from build123d import *

# Parameters (mm, degrees)
SKETCH1_W                                            = 120
SKETCH1_H                                            = 45
BOSS_EXTRUDE1_DEPTH                                  = 12
CHAMFER1_SIZE                                        = 1
SKETCH2_R                                            = 18
CUT_EXTRUDE1_DEPTH                                   = 66.193941436
M4_TAPPED_HOLE1_D                                    = 3.3
HOLE_SIZE_PER_SOCKET_HEAD_CAP_SCREW_TYPE_D           = 6.6
HOLE_SIZE_PER_SOCKET_HEAD_CAP_SCREW_TYPE_CBORE_D     = 11
HOLE_SIZE_PER_SOCKET_HEAD_CAP_SCREW_TYPE_CBORE_DEPTH = 6.8
SKETCH7_R                                            = 6
CUT_EXTRUDE2_DEPTH                                   = 3.2
M4_TAPPED_HOLE2_D                                    = 3.3
M4_TAPPED_HOLE2_DEPTH                                = 11.5
M4_TAPPED_HOLE2_TIP                                  = 0.991420021
M6_TAPPED_HOLE1_D                                    = 5


with BuildPart() as part:
    # Sketch1 → Boss-Extrude1 (new body)
    with BuildSketch(Plane(origin=(0, 0, 0), x_dir=(1, 0, 0), z_dir=(0, 1, 0))):
        Rectangle(SKETCH1_W, SKETCH1_H)
    extrude(amount=BOSS_EXTRUDE1_DEPTH)

    # Chamfer1
    chamfer1_edges = [part.edges().sort_by_distance(p)[0] for p in [
        (-60, 6, -22.5),
        (60, 6, -22.5),
        (60, 6, 22.5),
        (-60, 6, 22.5),
    ]]
    chamfer(chamfer1_edges, length=CHAMFER1_SIZE)

    # Sketch2 → Cut-Extrude1 (cut, through all)
    with BuildSketch(Plane(origin=(0, 12, 0), x_dir=(1, 0, 0), z_dir=(0, 1, 0))):
        with Locations(Location((0, 0, 0), (0, 0, 270))):
            Circle(SKETCH2_R)
    extrude(amount=-CUT_EXTRUDE1_DEPTH, mode=Mode.SUBTRACT)

    # M4 Tapped Hole1 (through all)
    with Locations(Plane(origin=(0, 12, 0), x_dir=(-1, 0, 0), z_dir=(0, 1, 0))):
        with Locations((15.5565, -15.5565), (15.5565, 15.5565), (-15.5565, 15.5565), (-15.5565, -15.5565)):
            Hole(M4_TAPPED_HOLE1_D / 2)

    # Hole size per socket head cap screw type1 (through all)
    with Locations(Plane(origin=(0, 12, 0), x_dir=(-1, 0, 0), z_dir=(0, 1, 0))):
        with Locations((51, 0), (-51, 0)):
            CounterBoreHole(HOLE_SIZE_PER_SOCKET_HEAD_CAP_SCREW_TYPE_D / 2, HOLE_SIZE_PER_SOCKET_HEAD_CAP_SCREW_TYPE_CBORE_D / 2, HOLE_SIZE_PER_SOCKET_HEAD_CAP_SCREW_TYPE_CBORE_DEPTH)

    # Sketch7 → Cut-Extrude2 (cut)
    with BuildSketch(Plane.XZ):
        with Locations(Location((51, 0, 0), (0, 0, 270))):
            Circle(SKETCH7_R)
        with Locations(Location((-51, 0, 0), (0, 0, 270))):
            Circle(SKETCH7_R)
    extrude(amount=-CUT_EXTRUDE2_DEPTH, mode=Mode.SUBTRACT)

    # M4 Tapped Hole2
    with Locations(Plane(origin=(0, 0, -22.5), x_dir=(-1, 0, 0), z_dir=(0, 0, -1))):
        with Locations((-27.5, 7)):
            Hole(M4_TAPPED_HOLE2_D / 2, depth=M4_TAPPED_HOLE2_DEPTH)
            with Locations((0, 0, -(M4_TAPPED_HOLE2_DEPTH + M4_TAPPED_HOLE2_TIP / 2))):  # 118° drill point
                Cone(0, M4_TAPPED_HOLE2_D / 2, M4_TAPPED_HOLE2_TIP, mode=Mode.SUBTRACT)

    # M6 Tapped Hole1 (through all)
    with Locations(Plane(origin=(0, 12, 0), x_dir=(1, 0, 0), z_dir=(0, 1, 0))):
        with Locations((35, -15), (35, 15), (-35, -15), (-35, 15)):
            Hole(M6_TAPPED_HOLE1_D / 2)


solid = part.part
Can you work these out from the model? Positions are in its coordinate system, mm. A direction names the side the tool comes from. Round coordinates to 2 decimals unless told otherwise and drop trailing zeros. Write each loop counter-clockwise with the first axis right and the second up, starting at its lowest first coordinate (ties: lowest second). Pieces come first, ordered by that corner, then holes. Notation, with made-up numbers: M 26.25,-35 L 63.25,-35 A24 ccw 63.25,1 Z; hole C -22,16.5 d11. An arc over 180 degrees is marked long. Use CSV: the item, a comma, the result in double quotes.
(1) Imagine slicing it at C-C (z = 0). Count the separate pieces of the cut face and the enclosed holes in it, plus the area to 3 significant figures.
Check values:
separate pieces,"4"
enclosed holes,"0"
area,"755 mm^2"
(2) Imagine slicing it at B-B (x = 35). Write out the boundary of the cut face in (y, z).
Check values:
outline,"M 0,-22.5 L 12,-22.5 L 12,-17.5 L 0,-17.5 Z; M 0,-12.5 L 12,-12.5 L 12,12.5 L 0,12.5 Z; M 0,17.5 L 12,17.5 L 12,22.5 L 0,22.5 Z"
(3) I need wall thicknesses on line 1 along X through (y, z) = (0.85, 0); line 2 along Z through (x, y) = (-35, 5); line 3 along X through (y, z) = (3.75, 16). Which ranges of each line are inside material? Lowest first, please.
Check values:
line 1,"-60 to -57, -45 to -18, 18 to 45, 57 to 60"
line 2,"-22.5 to -17.5, -12.5 to 12.5, 17.5 to 22.5"
line 3,"-60 to -37.29, -32.71 to -17.15, -13.97 to -8.25, 8.25 to 13.97, 17.15 to 32.71, 37.29 to 60"
(4) Imagine slicing it at D-D (x = 9). Write out the boundary of the cut face in (y, z).
Check values:
outline,"M 0,-22.5 L 12,-22.5 L 12,-15.59 L 0,-15.59 Z; M 0,15.59 L 12,15.59 L 12,22.5 L 0,22.5 Z"
(5) I'm going to push a flat-ended pin straight in: pin 1 (10 mm diameter, centred on x = 51, z = 0, fed in from -Y). Where does the tip first touch, or does it pass through?
Check values:
pin 1,"y = 3.2"
(6) Imagine slicing it at A-A (x = -51). Write out the boundary of the cut face in (y, z), plus the area to 3 significant figures.
Check values:
outline,"M 0,-22.5 L 12,-22.5 L 12,-5.5 L 5.2,-5.5 L 5.2,-3.3 L 3.2,-3.3 L 3.2,-6 L 0,-6 Z; M 0,6 L 3.2,6 L 3.2,3.3 L 5.2,3.3 L 5.2,5.5 L 12,5.5 L 12,22.5 L 0,22.5 Z"
area,"414 mm^2"
(7) On a 3-axis mill with a long thin cutter (end or side, diameter ignored), from which of +Z, -Z, +X, -X, +Y, -Y can I reach the whole of each face in a straight line? I mean faces 5 (the cylindrical face through (-14.032, 5.916, -16.188)), 6 (the flat face through (48, 3.2, -3)), 7 (the flat face through (51, 5.2, -4)). Say none if no direction works.
Check values:
face 5,"+Y, -Y"
face 6,"-Y"
face 7,"+Y"
(8) We'd pull the mould along Z, two halves only. Please class faces 1 (the conical face through (27.786, 7.013, -10.181)), 2 (the flat face through (-60, 6, 0)), 3 (the cylindrical face through (5.407, 6.084, 17.169)), 4 (the cylindrical face through (-49.198, 1.578, -5.723)): +Z half, -Z half, draft (parallel to the pull), parting line (faces both ways), or undercut.
Check values:
face 1,"-Z half"
face 2,"draft"
face 3,"undercut"
face 4,"undercut"
